Verification items for the finished model (mm, model axes). A direction names the side the tool comes from. Coordinates: 2 decimals unless noted, no trailing zeros. Loops run counter-clockwise (first coordinate to the right, second up) from the corner with the lowest first, then second, coordinate; pieces in that order, holes last. Notation, with made-up numbers: (-30, 79) -> (-23, 79) arc R17 ccw to (-23, 110) -> close; hole circle Ø2 at (88, 40.5). An arc over 180 degrees is marked (long way). Write item = value, one per line.
```python
from build123d import *

# Parameters (mm, degrees)
SKETCH_1_R      = 1.65
EXTRUDE_1_DEPTH = 12.25


with BuildPart() as part:
    # 草图1 → 凸台-拉伸1 (new body)
    with BuildSketch(Plane(origin=(0, 0, 0), x_dir=(1, 0, 0), z_dir=(0, 1, 0))):
        with BuildLine():
            Line((-24, -11), (-24, 11))
            ThreePointArc((-24, 11), (-23.121320344, 13.121320344), (-21, 14))
            Line((-21, 14), (21, 14))
            ThreePointArc((21, 14), (23.121320344, 13.121320344), (24, 11))
            Line((24, 11), (24, -11))
            ThreePointArc((24, -11), (23.121320344, -13.121320344), (21, -14))
            Line((21, -14), (-21, -14))
            ThreePointArc((-21, -14), (-23.121320344, -13.121320344), (-24, -11))
        make_face()
        with Locations(Location((-20, 10, 0), (0, 0, 270))):
            Circle(SKETCH_1_R, mode=Mode.SUBTRACT)
        with Locations(Location((-20, -10, 0), (0, 0, 270))):
            Circle(SKETCH_1_R, mode=Mode.SUBTRACT)
        with Locations(Location((20, -10, 0), (0, 0, 270))):
            Circle(SKETCH_1_R, mode=Mode.SUBTRACT)
        with Locations(Location((20, 10, 0), (0, 0, 270))):
            Circle(SKETCH_1_R, mode=Mode.SUBTRACT)
        with BuildLine():
            Line((-17, -4), (-17, 4))
            ThreePointArc((-17, 4), (-16.121320344, 6.121320344), (-14, 7))
            Line((-14, 7), (14, 7))
            ThreePointArc((14, 7), (16.121320344, 6.121320344), (17, 4))
            Line((17, 4), (17, -4))
            ThreePointArc((17, -4), (16.121320344, -6.121320344), (14, -7))
            Line((14, -7), (-14, -7))
            ThreePointArc((-14, -7), (-16.121320344, -6.121320344), (-17, -4))
        make_face(mode=Mode.SUBTRACT)
    extrude(amount=EXTRUDE_1_DEPTH)


solid = part.part
```
1) Sectioned sample at B-B, the plane x = 2. Record the cut outline in (y, z), plus the area to 4 significant figures.
Ans:
outline = (0, -14) -> (12.25, -14) -> (12.25, -7) -> (0, -7) -> close; (0, 7) -> (12.25, 7) -> (12.25, 14) -> (0, 14) -> close
area = 171.5 mm2
2) Sectioned sample at C-C, the plane z = 1.25. Record the cut outline in (x, y), plus the area to 4 significant figures.
Ans:
outline = (-24, 0) -> (-17, 0) -> (-17, 12.25) -> (-24, 12.25) -> close; (17, 0) -> (24, 0) -> (24, 12.25) -> (17, 12.25) -> close
area = 171.5 mm2
3) Tool access check on faces 5 (the face through (0, 6, 7)), 6 (the face through (-24, 6, 0)). Record the directions out of +Z, -Z, +X, -X, +Y, -Y that give a thin tool (end or side, any length) a straight path to the whole face; none if there is none.
Ans:
face_5 = +Y, -Y
face_6 = +Z, -Z, -X, +Y, -Y
4) Release check for a two-part mould opening along X. For faces 1 (the face through (24, 6, 0)), 2 (the face through (-23.1, 6.04, 13.14)), 3 (the face through (0, 6, 14)), 4 (the face through (-16.1, 6.04, 6.14)) record: pulls with the +X half, pulls with the -X half, needs draft (parallel to the pull), parting line crosses it, or undercut.
Ans:
face_1 = pulls with the +X half
face_2 = pulls with the -X half
face_3 = needs draft
face_4 = undercut
5) Material ranges on line 1 (X direction, y = 8.75, z = -10); line 2 (Z direction, x = 2, y = 0.75); line 3 (X direction, y = 10.5, z = -3.75), recorded low to high.
Ans:
line_1 = -24 to -21.65, -18.35 to 18.35, 21.65 to 24
line_2 = -14 to -7, 7 to 14
line_3 = -24 to -17, 17 to 24
6) Sectioned sample at A-A, the plane x = -20. Record the cut outline in (y, z).
Ans:
outline = (0, -14) -> (12.25, -14) -> (12.25, -11.65) -> (0, -11.65) -> close; (0, -8.35) -> (12.25, -8.35) -> (12.25, 8.35) -> (0, 8.35) -> close; (0, 11.65) -> (12.25, 11.65) -> (12.25, 14) -> (0, 14) -> close
7) Sectioned sample at D-D, the plane y = 3.75. Record the cut outline in (x, z), plus the area to 3 significant figures.
Ans:
outline = (-24, -11) arc R3 ccw to (-21, -14) -> (21, -14) arc R3 ccw to (24, -11) -> (24, 11) arc R3 ccw to (21, 14) -> (-21, 14) arc R3 ccw to (-24, 11) -> close; hole circle Ø3.3 at (-20, -10); hole circle Ø3.3 at (-20, 10); hole (-17, -4) arc R3 ccw to (-14, -7) -> (14, -7) arc R3 ccw to (17, -4) -> (17, 4) arc R3 ccw to (14, 7) -> (-14, 7) arc R3 ccw to (-17, 4) -> close; hole circle Ø3.3 at (20, -10); hole circle Ø3.3 at (20, 10)
area = 834 mm2
